For this review, take the finished solid that the model builds, in its own axes (mm). Coordinates: 2 decimals unless noted, no trailing zeros. Write each loop counter-clockwise with the first axis right and the second up, starting at its lowest first coordinate (ties: lowest second). Pieces come first, ordered by that corner, then holes.
```python
from build123d import *

# Parameters (mm, degrees)
SKETCH1_R           = 8
BOSS_EXTRUDE1_DEPTH = 10


with BuildPart() as part:
    # Sketch1 → Boss-Extrude1 (new body)
    with BuildSketch(Plane.XY):
        Polygon((5137.305231976, 2244.717137192), (5129.46700669, 2304.202952513), (5169.124216904, 2309.428436037), (5184.800667476, 2190.456805396), (5145.143457262, 2185.231321872), align=None)
        with Locations((5151.908353559, 2286.987089168)):
            Circle(SKETCH1_R, mode=Mode.SUBTRACT)
        with Locations(Location((5162.359320607, 2207.67266874, 0), (0, 0, 180))):
            Circle(SKETCH1_R, mode=Mode.SUBTRACT)
    extrude(amount=BOSS_EXTRUDE1_DEPTH)


solid = part.part
```
Q1. Add section C-C (z = 7.5). State the section outline as (x, y) points.
Ans:
outline: (5129.47, 2304.2) - (5145.14, 2185.23) - (5184.8, 2190.46) - (5169.12, 2309.43) - close; hole circle Ø16 at (5151.91, 2286.99); hole circle Ø16 at (5162.36, 2207.67)
Q2. Add section A-A (x = 5148). State the section outline as (y, z) points.
Ans:
outline: (2185.61, 0) - (2280.01, 0) - (2280.01, 10) - (2185.61, 10) - close; (2293.97, 0) - (2306.64, 0) - (2306.64, 10) - (2293.97, 10) - close
Q3. Add section B-B (y = 2293.5). State the section outline as (x, z) points.
Ans:
outline: (5130.88, 0) - (5147.26, 0) - (5147.26, 10) - (5130.88, 10) - close; (5156.55, 0) - (5171.22, 0) - (5171.22, 10) - (5156.55, 10) - close
Q4. Clearance check with flat-ended pins moving along their axes: pin 1 Ø14.5 at (x, y) = (5151.91, 2286.99) entering from +Z; pin 2 Ø2 at (y, z) = (2237.5, 7) entering from +X; pin 3 Ø2 at (y, z) = (2206.5, 3) entering from +X; pin 4 Ø1 at (y, z) = (2270, 5.5) entering from +X. State where each tip first meets the part, or that it passes through.
Ans:
pin 1: passes through
pin 2: stops at x = 5178.73
pin 3: stops at x = 5182.82
pin 4: stops at x = 5174.39
Q5. Add section D-D (x = 5174.5). State the section outline as (y, z) points, then the cut area to 3 significant figures.
Ans:
outline: (2189.1, 0) - (2268.63, 0) - (2268.63, 10) - (2189.1, 10) - close
area: 795 mm2
Q6. For probe 1 along Y at (x, z) = (5168, 2.5); probe 2 along Y at (x, z) = (5153.5, 9.5); probe 3 along X at (y, z) = (2208, 7.5), list the stretches that pass through material, from the lowest coordinate up.
Ans:
probe 1: y = 2188.24 to 2202, 2213.35 to 2309.28
probe 2: y = 2186.33 to 2279.15, 2294.83 to 2307.37
probe 3: x = 5142.14 to 5154.37, 5170.35 to 5182.49
Q7. Draft analysis for pull direction X (two halves, no side actions). For faces 1 (the flat face through (5149.02, 2306.78, 4.93)), 2 (the cylindrical face through (5150.87, 2294.92, 4.93)), 3 (the flat face through (5165.25, 2187.88, 4.93)), state which applies: +X half, -X half, draft (parallel to the pull), parting line (faces both ways), or undercut.
Ans:
face 1: -X half
face 2: undercut
face 3: +X half
